from build123d import *

# Parameters (mm, degrees)
SKETCH1_W           = 50
SKETCH1_H           = 85
BOSS_EXTRUDE1_DEPTH = 6
SKETCH2_W           = 18
SKETCH2_H           = 14.448315912
BOSS_EXTRUDE2_DEPTH = 16
FILLET1_R           = 5
SKETCH3_W           = 6
SKETCH3_H           = 29.716496746
CUT_EXTRUDE1_DEPTH  = 16
SKETCH4_R           = 3
CUT_EXTRUDE2_DEPTH  = 95.154128959


with BuildPart() as part:
    # Sketch1 → Boss-Extrude1 (new body)
    with BuildSketch(Plane.XY):
        with Locations((25, 42.5)):
            Rectangle(SKETCH1_W, SKETCH1_H)
    extrude(amount=BOSS_EXTRUDE1_DEPTH)

    # Sketch2 → Boss-Extrude2 (add)
    with BuildSketch(Plane.XY.offset(6)):
        with Locations((25, 42.5)):
            Rectangle(SKETCH2_W, SKETCH2_H)
    extrude(amount=BOSS_EXTRUDE2_DEPTH)

    # Fillet1
    fillet1_edges = [part.edges().sort_by_distance(p)[0] for p in [
        (50, 42.5, 6),
        (25, 85, 6),
        (0, 42.5, 6),
        (25, 0, 6),
    ]]
    fillet(fillet1_edges, radius=FILLET1_R)

    # Sketch3 → Cut-Extrude1 (cut)
    with BuildSketch(Plane.XY.offset(22)):
        with Locations((25, 34.711959109)):
            Rectangle(SKETCH3_W, SKETCH3_H)
    extrude(amount=-CUT_EXTRUDE1_DEPTH, mode=Mode.SUBTRACT)

    # Sketch4 → Cut-Extrude2 (cut, through all)
    with BuildSketch(Plane.ZY.offset(-16)):
        with Locations(Location((14.673320443, 42.507843144, 0), (0, 0, 270))):
            Circle(SKETCH4_R)
        with BuildLine():
            Line((14.673320443, 49.895764166), (20.802104858, 55.115800091))
            Line((20.802104858, 55.115800091), (35.798114719, 48.402784846))
            Line((35.798114719, 48.402784846), (20.212830652, 12.710723094))
            Line((20.212830652, 12.710723094), (14.673320443, 35.119922122))
            ThreePointArc((14.673320443, 35.119922122), (22.061241465, 42.507843144), (14.673320443, 49.895764166))
        make_face()
    extrude(amount=-CUT_EXTRUDE2_DEPTH, mode=Mode.SUBTRACT)


solid = part.part
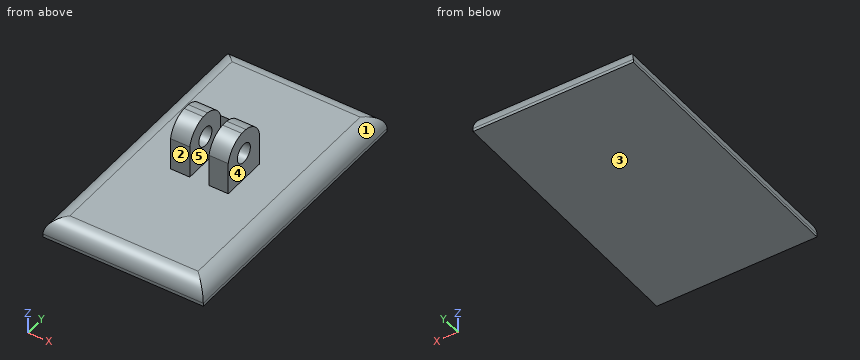
Check sheet for the modelled part. Datum: model origin and axes. Units: mm. Face numbers are marked on the shaded views. A direction names the side the tool comes from. Give positions to 0.01 mm unless a question says otherwise; leave off trailing zeros. Write each loop counter-clockwise with the first axis right and the second up, starting at its lowest first coordinate (ties: lowest second). Pieces come first, ordered by that corner, then holes. Notation, with made-up numbers: M 60.5,-35.5 L 93.5,-35.5 A23 cw 93.5,-10.5 Z; hole C 84,-20 d4. An arc over 180 degrees is marked long. Use one line per item in the form item = value.
(1) Section check A-A on z = 12.75. Record the boundary of the cut face in (x, y), plus the area to 3 significant figures.
Answer block:
outline = M 16,35.28 L 22,35.28 L 22,40.21 L 16,40.21 Z; M 16,44.81 L 22,44.81 L 22,49.57 L 28,49.57 L 28,44.81 L 34,44.81 L 34,49.72 L 16,49.72 Z; M 28,35.28 L 34,35.28 L 34,40.21 L 28,40.21 Z
area = 119 mm2
(2) Section check C-C on y = 26. Record the boundary of the cut face in (x, z).
Answer block:
outline = M 0,0 L 50,0 L 50,1 A5 ccw 45,6 L 5,6 A5 ccw 0,1 Z
(3) Material ranges on line 1 along Z through (x, y) = (27, 75); line 2 along Y through (x, z) = (32.5, 9.25); line 3 along X through (y, z) = (48, 4), recorded low to high.
Answer block:
line_1 = 0 to 6
line_2 = 35.28 to 49.72
line_3 = 1 to 49
(4) Section check D-D on x = 18. Record the boundary of the cut face in (y, z), plus the area to 3 significant figures.
Answer block:
outline = M 0,0 L 85,0 L 85,1 A5 ccw 80,6 L 49.72,6 L 49.72,16.26 A7.39 ccw 43.46,22 L 41.56,22 A7.39 ccw 35.28,16.18 L 35.28,6 L 5,6 A5 ccw 0,1 Z; hole C 42.51,14.67 d6
area = 682 mm2
(5) Depth check by flat-ended pin: P1, Ø7, axis at y = 42.51, z = 14.67, coming from the -X side; P2, Ø5, axis at x = 20.5, y = 19.5, coming from the +Z side; P3, Ø10, axis at x = 27.5, z = 7, coming from the -Y side. Enter the tip coordinate at first touch or a pass-through.
Answer block:
P1 = 16
P2 = 6
P3 = 0.1
(6) Tool access check on the marked faces 1 and 2. Record the directions out of +Z, -Z, +X, -X, +Y, -Y that give a thin tool (end or side, any length) a straight path to the whole face; none if there is none.
Answer block:
face_1 = +Z, +X, +Y, -Y
face_2 = +Z, +X, -X, -Y
(7) Section check B-B on x = 9. Record the boundary of the cut face in (y, z).
Answer block:
outline = M 0,0 L 85,0 L 85,1 A5 ccw 80,6 L 5,6 A5 ccw 0,1 Z
(8) Draft check along X on the marked faces 3, 4 and 5. Enter one of: pulls with the +X half, pulls with the -X half, needs draft (parallel to the pull), parting line crosses it, or undercut.
Answer block:
face_3 = needs draft
face_4 = pulls with the +X half
face_5 = undercut
